Design review of the part built by this model. Coordinates are the model's own, in mm. Give positions to 0.01 mm unless a question says otherwise; leave off trailing zeros. Write each loop counter-clockwise with the first axis right and the second up, starting at its lowest first coordinate (ties: lowest second). Pieces come first, ordered by that corner, then holes. Notation, with made-up numbers: M -33,54 L 2,54 A16 cw 2,79 Z; hole C 43,70.5 d6. An arc over 180 degrees is marked long. Use one line per item in the form item = value. Start each with the question number.
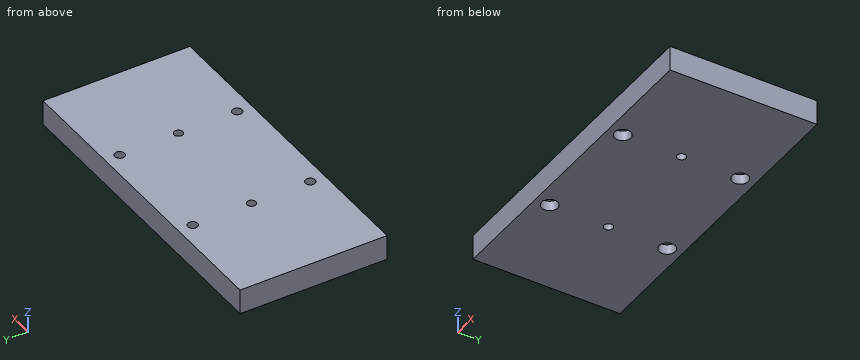
from build123d import *

# Parameters (mm, degrees)
SKETCH1_W                               = 216
SKETCH1_H                               = 100
BOSS_EXTRUDE1_DEPTH                     = 17
F_6_0_6_DIAMETER_HOLE1_D                = 6
CBORE_FOR_M6_HEX_HEAD_BOLT1_D           = 6.6
CBORE_FOR_M6_HEX_HEAD_BOLT1_CBORE_D     = 11
CBORE_FOR_M6_HEX_HEAD_BOLT1_CBORE_DEPTH = 6.8


with BuildPart() as part:
    # Sketch1 → Boss-Extrude1 (new body)
    with BuildSketch(Plane(origin=(0, 0, 0), x_dir=(-1, 0, 0), z_dir=(0, 0, -1))):
        Rectangle(SKETCH1_W, SKETCH1_H)
    extrude(amount=-BOSS_EXTRUDE1_DEPTH)

    # Ø6.0 (6) Diameter Hole1 (through all)
    with Locations(Plane(origin=(0, 0, 0), x_dir=(-1, 0, 0), z_dir=(0, 0, -1))):
        with Locations((-40, 0), (40, 0)):
            Hole(F_6_0_6_DIAMETER_HOLE1_D / 2)

    # CBORE for M6 Hex Head Bolt1 (through all)
    with Locations(Plane(origin=(0, 0, 0), x_dir=(-1, 0, 0), z_dir=(0, 0, -1))):
        with Locations((40, 40), (40, -40), (-40, -40), (-40, 40)):
            CounterBoreHole(CBORE_FOR_M6_HEX_HEAD_BOLT1_D / 2, CBORE_FOR_M6_HEX_HEAD_BOLT1_CBORE_D / 2, CBORE_FOR_M6_HEX_HEAD_BOLT1_CBORE_DEPTH)


solid = part.part
1. Clearance check with a flat-ended pin moving along its axis: pin 1 Ø7.5 at (x, y) = (40, 40) entering from -Z. State where the tip first meets the part, or that it passes through.
2. We need section A-A (y = -40). State the section outline as (x, z) points.
3. We need section C-C (z = 2). State the section outline as (x, y) points.
4. We need section B-B (x = -40). State the section outline as (y, z) points, and give its area (3 significant figures).
5. To check wall thickness, follow L1, parallel to Y at x = 40, z = 14.25; L2, parallel to Y at x = -40, z = 4.75; L3, parallel to X at y = -37.5, z = 12.75. State the ranges of each line that lie inside material, in increasing order.
Answer block:
q1.pin_1 = 6.8
q2.outline = M -108,0 L -45.5,0 L -45.5,6.8 L -43.3,6.8 L -43.3,17 L -108,17 Z; M -36.7,6.8 L -34.5,6.8 L -34.5,0 L 34.5,0 L 34.5,6.8 L 36.7,6.8 L 36.7,17 L -36.7,17 Z; M 43.3,6.8 L 45.5,6.8 L 45.5,0 L 108,0 L 108,17 L 43.3,17 Z
q3.outline = M -108,-50 L 108,-50 L 108,50 L -108,50 Z; hole C -40,-40 d11; hole C -40,40 d11; hole C -40,0 d6; hole C 40,-40 d11; hole C 40,40 d11; hole C 40,0 d6
q4.outline = M -50,0 L -45.5,0 L -45.5,6.8 L -43.3,6.8 L -43.3,17 L -50,17 Z; M -36.7,6.8 L -34.5,6.8 L -34.5,0 L -3,0 L -3,17 L -36.7,17 Z; M 3,0 L 34.5,0 L 34.5,6.8 L 36.7,6.8 L 36.7,17 L 3,17 Z; M 43.3,6.8 L 45.5,6.8 L 45.5,0 L 50,0 L 50,17 L 43.3,17 Z
q4.area = 1,310 mm^2
q5.L1 = -50 to -43.3, -36.7 to -3, 3 to 36.7, 43.3 to 50
q5.L2 = -50 to -45.5, -34.5 to -3, 3 to 34.5, 45.5 to 50
q5.L3 = -108 to -42.15, -37.85 to 37.85, 42.15 to 108
